The model under review builds one solid part; all positions refer to its coordinate system, in mm. Round coordinates to 2 decimals unless told otherwise and drop trailing zeros. Order: outer loops, then holes, each group sorted by start corner. A loop starts at its lowest first (then second) coordinate and runs counter-clockwise, first axis right, second up. Notation, with made-up numbers: M -21.5,11.5 L -12.5,11.5 A13 cw -12.5,18.5 Z; hole C 48,20.5 d9. An arc over 180 degrees is marked long. Answer as a JSON object with one key per item and string values. Group by question number.
1) To check wall thickness, follow line 1 (X direction, y = 5.5, z = -3.25); line 2 (Y direction, x = 61.5, z = -1.5). State the ranges of each line that lie inside material, in increasing order.
2) Consider section C-C, the plane x = 9.5. Write out the cut boundary in (y, z), then the cut area to 3 significant figures.
3) Insertion check: pin 1 Ø6 at (y, z) = (4.5, -4) entering from -X; pin 2 Ø3 at (x, z) = (84.5, -3) entering from -Y. Each pin has a flat end and moves straight along its axis. Give the tip position at first contact, or say it passes through.
4) Consider section A-A, the plane y = 0. Write out the cut boundary in (x, z) (1 decimal), then the cut area to 3 significant figures.
```python
from build123d import *


with BuildPart() as part:
    # Sketch1 → Revolve1 (revolve)
    with BuildSketch(Plane(origin=(0, 0, 0), x_dir=(-1, 0, 0), z_dir=(0, 0, -1)), mode=Mode.PRIVATE) as revolve1_sk:
        Polygon((-135.5, 8), (-135.5, 0), (28, 0), (28, 2.0095), (27.5095, 2.5), (13, 2.5), (13, 2.065), (11.5, 2.065), (11.5, 2.5), (-130.5, 2.5), (-130.5, 8), align=None)
    revolve(revolve1_sk.sketch.rotate(Axis((135.5, 0, 0), (-1, 0, 0)), 270), axis=Axis((135.5, 0, 0), (-1, 0, 0)))


solid = part.part
```
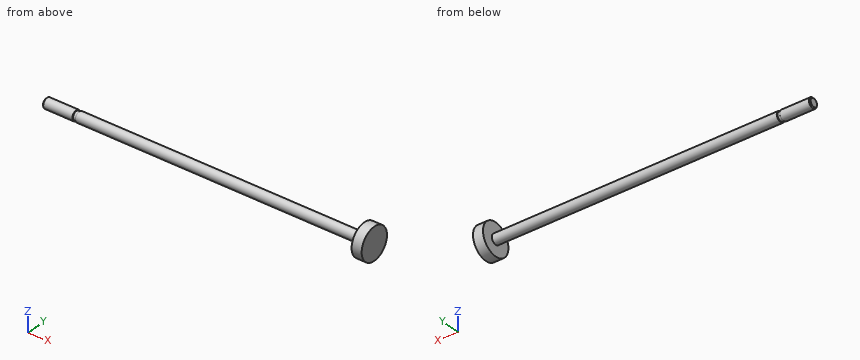
Results list:
{
 "1": {"line 1": "130.5 to 135.5", "line 2": "-2 to 2"},
 "2": {"outline": "C 0,0 d5", "area": "19.6 mm^2"},
 "3": {"pin 1": "x = 130.5", "pin 2": "y = -2"},
 "4": {"outline": "M -28,-2 L -27.5,-2.5 L -13,-2.5 L -13,-2.1 L -11.5,-2.1 L -11.5,-2.5 L 130.5,-2.5 L 130.5,-8 L 135.5,-8 L 135.5,8 L 130.5,8 L 130.5,2.5 L -11.5,2.5 L -11.5,2.1 L -13,2.1 L -13,2.5 L -27.5,2.5 L -28,2 Z", "area": "871 mm^2"}
}
